```python
from build123d import *

# Parameters (mm, degrees)
SKETCH_1_W             = 8
SKETCH_1_H             = 196
HOLE_WIZARD_M8_1_D     = 6.8
HOLE_WIZARD_M8_1_DEPTH = 8
HOLE_WIZARD_M8_1_TIP   = 2.042926105
HOLE_WIZARD_M8_2_D     = 6.8
HOLE_WIZARD_M8_2_DEPTH = 8
HOLE_WIZARD_M8_2_TIP   = 2.042926105


with BuildPart() as part:
    # 草图1 → 旋转-薄壁1 (revolve)
    with BuildSketch(Plane.XY, mode=Mode.PRIVATE) as revolve_1_sk:
        with Locations((-4, 98)):
            Rectangle(SKETCH_1_W, SKETCH_1_H)
    revolve(revolve_1_sk.sketch.rotate(Axis((0, 0, 0), (0, 1, 0)), 270), axis=Axis((0, 0, 0), (0, 1, 0)))

    # M8 螺纹孔的螺纹孔钻头1
    with Locations(Plane(origin=(0, 0, 0), x_dir=(-1, 0, 0), z_dir=(0, -1, 0))):
        with Locations((0, 0)):
            Hole(HOLE_WIZARD_M8_1_D / 2, depth=HOLE_WIZARD_M8_1_DEPTH)
            with Locations((0, 0, -(HOLE_WIZARD_M8_1_DEPTH + HOLE_WIZARD_M8_1_TIP / 2))):  # 118° drill point
                Cone(0, HOLE_WIZARD_M8_1_D / 2, HOLE_WIZARD_M8_1_TIP, mode=Mode.SUBTRACT)

    # M8 螺纹孔的螺纹孔钻头2
    with Locations(Plane(origin=(0, 196, 0), x_dir=(1, 0, 0), z_dir=(0, 1, 0))):
        with Locations((0, 0)):
            Hole(HOLE_WIZARD_M8_2_D / 2, depth=HOLE_WIZARD_M8_2_DEPTH)
            with Locations((0, 0, -(HOLE_WIZARD_M8_2_DEPTH + HOLE_WIZARD_M8_2_TIP / 2))):  # 118° drill point
                Cone(0, HOLE_WIZARD_M8_2_D / 2, HOLE_WIZARD_M8_2_TIP, mode=Mode.SUBTRACT)


solid = part.part
```
Verification items for the finished model (mm, model axes). A direction names the side the tool comes from. Round coordinates to 2 decimals unless told otherwise and drop trailing zeros. Write each loop counter-clockwise with the first axis right and the second up, starting at its lowest first coordinate (ties: lowest second). Pieces come first, ordered by that corner, then holes.
1. Scan lines: L1, parallel to Z at x = 1, y = 188; L2, parallel to X at y = 67, z = -0.5; L3, parallel to Z at x = -3.5, y = 140. Record each from-to range of solid material in increasing order.
2. Gauge pin test, flat ends, axial feed: P1, Ø6, axis at y = 134, z = -6, coming from the -X side; P2, Ø1.5, axis at x = 6, y = 93, coming from the -Z side; P3, Ø6, axis at x = 0, z = 0, coming from the +Y side. Record the tip position at first contact, or that the pin passes through.
3. Section check A-A on y = 28. Enter the section's corners in (x, z).
4. Section check B-B on x = 5.75. Enter the section's corners in (y, z), plus the area to 3 significant figures.
5. Draft check along Z on faces 4 (the cylindrical face through (7.81, 99.37, 1.73)), 5 (the conical face through (0.128, 9.688, 0.576)), 6 (the flat face through (2, 196, -3)), 7 (the conical face through (-0.128, 186.312, 0.576)). Enter one of: +Z half, -Z half, draft (parallel to the pull), parting line (faces both ways), or undercut.
6. Access from +Z, -Z, +X, -X, +Y, -Y to the whole of each face (thin tool, end or side, straight path). Record for faces 1 (the flat face through (2, 0, -3)), 2 (the cylindrical face through (0.74, 191.94, 3.32)), 3 (the cylindrical face through (-0.74, 4.06, 3.32)).
Answer:
1. L1: z = -7.94 to -3.25, 3.25 to 7.94
1. L2: x = -7.98 to 7.98
1. L3: z = -7.19 to 7.19
2. P1: stops at x = -7.42
2. P2: stops at z = -6.04
2. P3: stops at y = 187.76
3. outline: circle Ø16 at (0, 0)
4. outline: (0, -5.56) - (196, -5.56) - (196, 5.56) - (0, 5.56) - close
4. area: 2,180 mm2
5. face 4: parting line
5. face 5: undercut
5. face 6: draft
5. face 7: undercut
6. face 1: +Z, -Z, +X, -X, -Y
6. face 2: +Y
6. face 3: -Y
